Could you check a few things on this model? Use its own coordinates, in mm. A direction names the side the tool comes from. Coordinates: 2 decimals unless noted, no trailing zeros. Write each loop counter-clockwise with the first axis right and the second up, starting at its lowest first coordinate (ties: lowest second). Pieces come first, ordered by that corner, then holes.
Item 1: Which directions (+Z, -Z, +X, -X, +Y, -Y) give clear straight access to the entire face, cutting with the end or side of a thin tool? Please do faces 4 (the flat face through (0, -197, -45)), 5 (the flat face through (0, 76, 0)).
Item 2: I want a section at D-D on z = 61. Please give me the cut outline in (x, y).
Item 3: Thinking about a two-plate mould opening in Z: for faces 1 (the cylindrical face through (0.1, -205.37, 16.19)), 2 (the flat face through (-7, -182, 12)), 3 (the flat face through (0, -139, 70)), which applies, +Z half, -Z half, draft (parallel to the pull), parting line (faces both ways), or undercut?
Item 4: If I drill on probe 1 along Y at (x, z) = (1.25, 15); probe 2 along Y at (x, z) = (5.5, -22); probe 3 along Z at (x, y) = (-2.5, 86.5), over which ranges is the centre line in solid material (lowest first)?
Item 5: I want a section at C-C on x = 2.75. Please give me the cut outline in (y, z), then the cut area to 3 significant figures.
Item 6: I want a section at A-A on z = 15. Please give me the cut outline in (x, y), then the cut area to 3 significant figures.
Item 7: I want a section at B-B on y = -200. Please give me the cut outline in (x, z).
from build123d import *

# Parameters (mm, degrees)
EXTRUDE_1_DEPTH     = 7
CUT_EXTRUDE_2_REACH = 408.32
SKETCH_3_R          = 5.5
CHAMFER_1_SIZE      = 20


with BuildPart() as part:
    # 草图1 → 凸台-拉伸1 (new, symmetric)
    with BuildSketch(Plane(origin=(0, 0, 0), x_dir=(0, 0, -1), z_dir=(1, 0, 0))):
        Polygon((0, 0), (45, 0), (45, -400), (-70, -400), (-70, 150), (0, 150), align=None)
    extrude(amount=EXTRUDE_1_DEPTH, both=True)

    # 草图3 → 切除-拉伸2 (cut, up to next)
    with BuildSketch(Plane(origin=(7, 0, 0), x_dir=(0, 0, -1), z_dir=(1, 0, 0)), mode=Mode.PRIVATE) as cut_extrude_2_sk1:
        with Locations((-15, -200)):
            Circle(SKETCH_3_R)
    cut_extrude_2_tool1 = extrude(cut_extrude_2_sk1.sketch, amount=-CUT_EXTRUDE_2_REACH, mode=Mode.PRIVATE) & part.part
    add(cut_extrude_2_tool1.solids().sort_by_distance((7, -200, 15))[0], mode=Mode.SUBTRACT)

    # 倒角1
    chamfer_1_edges = [part.edges().sort_by_distance(p)[0] for p in [
        (0, 150, 70),
    ]]
    chamfer(chamfer_1_edges, length=CHAMFER_1_SIZE)


solid = part.part
Response values:
1. face 4: -Z, +X, -X, +Y, -Y
1. face 5: -Z, +X, -X, +Y
2. outline: (-7, -400) - (7, -400) - (7, 139) - (-7, 139) - close
3. face 1: undercut
3. face 2: draft
3. face 3: +Z half
4. probe 1: y = -400 to -205.5, -194.5 to 150
4. probe 2: y = -400 to 0
4. probe 3: z = 0 to 70
5. outline: (-400, -45) - (0, -45) - (0, 0) - (150, 0) - (150, 50) - (130, 70) - (-400, 70) - close; hole circle Ø11 at (-200, 15)
5. area: 56,200 mm2
6. outline: (-7, -400) - (7, -400) - (7, -205.5) - (-7, -205.5) - close; (-7, -194.5) - (7, -194.5) - (7, 150) - (-7, 150) - close
6. area: 7,550 mm2
7. outline: (-7, -45) - (7, -45) - (7, 9.5) - (-7, 9.5) - close; (-7, 20.5) - (7, 20.5) - (7, 70) - (-7, 70) - close
